from build123d import *


with BuildPart() as part:
    # Sketch1 → Revolve1 (revolve)
    with BuildSketch(Plane.XY, mode=Mode.PRIVATE) as revolve1_sk:
        Polygon((0, 0), (80, 0), (80, 9.9), (110, 9.9), (110, 23.9), (107.5, 23.9), (107.5, 43.9), (110, 43.9), (110, 53.9), (99.5, 53.9), (99.5, 62), (110, 62), (110, 72), (107.5, 72), (107.5, 92), (110, 92), (110, 106), (80, 106), (80, 116), (65, 116), (65, 1698), (61.360297657, 1708), (30, 1708), (30, 1728), (0, 1728), align=None)
    revolve(revolve1_sk.sketch.rotate(Axis((0, 0, 0), (0, 1, 0)), 90), axis=Axis((0, 0, 0), (0, 1, 0)))


solid = part.part
Check sheet for the modelled part. Datum: model origin and axes. Units: mm. A direction names the side the tool comes from. Round coordinates to 2 decimals unless told otherwise and drop trailing zeros. Write each loop counter-clockwise with the first axis right and the second up, starting at its lowest first coordinate (ties: lowest second). Pieces come first, ordered by that corner, then holes. Notation, with made-up numbers: (34, 85.25) -> (90, 85.25) arc R20 ccw to (90, 103.25) -> close; hole circle Ø4 at (34.25, -0.75). An arc over 180 degrees is marked (long way). Answer as CSV lines item,"result". Start each with the question number.
1) Material ranges on line 1 (Y direction, x = -72, z = -77); line 2 (X direction, y = 1644, z = 22); line 3 (Z direction, x = 0.5, y = 511), recorded low to high. Write a range as from..to.
2) Tool access check on faces 4 (the flat face through (57, 62, -82)), 5 (the cylindrical face through (-3.517, 5.019, 79.923)), 6 (the cylindrical face through (-25.296, 1718.14, -16.128)). Record the directions out of +Z, -Z, +X, -X, +Y, -Y that give a thin tool (end or side, any length) a straight path to the whole face; none if there is none.
3) Release check for a two-part mould opening along Y. For faces 1 (the cylindrical face through (97.59, 67.07, -50.76)), 2 (the flat face through (-66, 116, 0)), 3 (the flat face through (105, 23.9, -24)) record: pulls with the +Y half, pulls with the -Y half, needs draft (parallel to the pull), parting line crosses it, or undercut.
4) Section check A-A on y = 1462. Enter the section's corners in (x, z), and give its area (3 significant figures).
5) Go/stop test with flat-tipped pins: P1, Ø1, axis at x = 33.5, y = 1346, coming from the +Z side; P2, Ø4, axis at x = -51, z = -50, coming from the +Y side; P3, Ø1.5, axis at x = -2.5, y = 641, coming from the +Z side. Record where each tip stops, or that it passes through.
Found:
1,line 1,"y = 9.9..53.9, 62..106"
1,line 2,"x = -61.16..61.16"
1,line 3,"z = -65..65"
2,face 4,"none"
2,face 5,"-Y"
2,face 6,"+Y"
3,face 1,"needs draft"
3,face 2,"pulls with the +Y half"
3,face 3,"undercut"
4,outline,"circle Ø130 at (0, 0)"
4,area,"13,300 mm^2"
5,P1,"stops at z = 56"
5,P2,"stops at y = 116"
5,P3,"stops at z = 64.98"
